```python
from build123d import *

# Parameters (mm, degrees)
SKETCH1_W           = 50
SKETCH1_H           = 18
BOSS_EXTRUDE1_DEPTH = 3
M5_TAPPED_HOLE1_D   = 4.2
CHAMFER1_SIZE       = 2


with BuildPart() as part:
    # Sketch1 → Boss-Extrude1 (new, symmetric)
    with BuildSketch(Plane.XY):
        Rectangle(SKETCH1_W, SKETCH1_H)
    extrude(amount=BOSS_EXTRUDE1_DEPTH, both=True)

    # M5 Tapped Hole1 (through all)
    with Locations(Plane.XY.offset(3)):
        with Locations((-17.5, 0), (17.5, 0)):
            Hole(M5_TAPPED_HOLE1_D / 2)

    # Chamfer1
    chamfer1_edges = [part.edges().sort_by_distance(p)[0] for p in [
        (-25, 9, 0),
        (25, 9, 0),
        (25, -9, 0),
        (-25, -9, 0),
    ]]
    chamfer(chamfer1_edges, length=CHAMFER1_SIZE)


solid = part.part
```
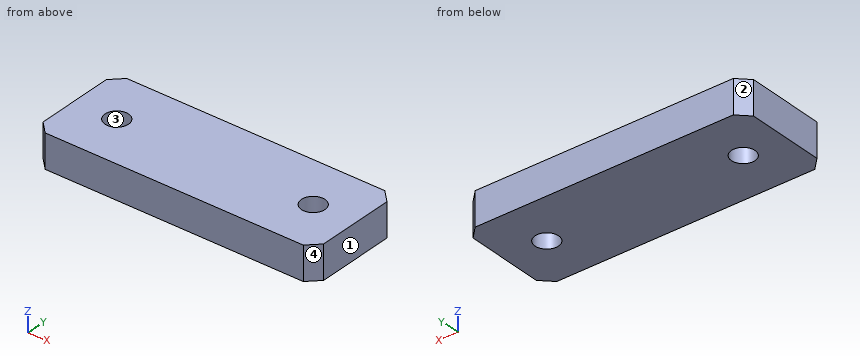
Read the model definition and answer for the solid it produces. Units are mm, in the model's axes. Face numbers are marked on the shaded views. Coordinates: 2 decimals unless noted, no trailing zeros. Write each loop counter-clockwise with the first axis right and the second up, starting at its lowest first coordinate (ties: lowest second). Pieces come first, ordered by that corner, then holes. Notation, with made-up numbers: (37.25, -12) -> (70.25, -12) arc R23 ccw to (70.25, 17) -> close; hole circle Ø10 at (65.25, -36.75). An arc over 180 degrees is marked (long way). Answer as a JSON object with one key per item and string values.
Q1. A flat-ended cylindrical pin translates along its axis: pin 1 Ø3.5 at (x, y) = (-17.5, 0) entering from +Z. Find the tip coordinate at first contact, or state that the pin passes through.
The answers:
{"pin 1": "passes through"}
Q2. Consider line 1 (Y direction, x = -17.5, z = -1.75); line 2 (X direction, y = -1.75, z = -2.2); line 3 (X direction, y = 0.5, z = 1.9). Determine where each line is inside the solid, lowest interval first. Write a range as [from, to].
The answers:
{"line 1": "y = [-9, -2.1], [2.1, 9]", "line 2": "x = [-25, -18.66], [-16.34, 16.34], [18.66, 25]", "line 3": "x = [-25, -19.54], [-15.46, 15.46], [19.54, 25]"}
Q3. The part is cut by section B-B on x = 17.5. Give the vertices of the cut face in (y, z).
The answers:
{"outline": "(-9, -3) -> (-2.1, -3) -> (-2.1, 3) -> (-9, 3) -> close; (2.1, -3) -> (9, -3) -> (9, 3) -> (2.1, 3) -> close"}
Q4. The part is cut by section A-A on y = 0. Give the vertices of the cut face in (x, z), then the cut area to 3 significant figures.
The answers:
{"outline": "(-25, -3) -> (-19.6, -3) -> (-19.6, 3) -> (-25, 3) -> close; (-15.4, -3) -> (15.4, -3) -> (15.4, 3) -> (-15.4, 3) -> close; (19.6, -3) -> (25, -3) -> (25, 3) -> (19.6, 3) -> close", "area": "250 mm2"}
Q5. Determine the mould class of the marked faces 1, 2, 3 and 4 for opening direction Y: pulls with the +Y half, pulls with the -Y half, needs draft (parallel to the pull), parting line crosses it, or undercut.
The answers:
{"face 1": "needs draft", "face 2": "pulls with the +Y half", "face 3": "undercut", "face 4": "pulls with the -Y half"}
Q6. The part is cut by section C-C on z = -0.9. Give the vertices of the cut face in (x, y), then the cut area to 3 significant figures.
The answers:
{"outline": "(-25, -7) -> (-23, -9) -> (23, -9) -> (25, -7) -> (25, 7) -> (23, 9) -> (-23, 9) -> (-25, 7) -> close; hole circle Ø4.2 at (-17.5, 0); hole circle Ø4.2 at (17.5, 0)", "area": "864 mm2"}
